Check sheet for the modelled part. Datum: model origin and axes. Units: mm. Face numbers are marked on the shaded views. A direction names the side the tool comes from. Round coordinates to 2 decimals unless told otherwise and drop trailing zeros. Write each loop counter-clockwise with the first axis right and the second up, starting at its lowest first coordinate (ties: lowest second). Pieces come first, ordered by that corner, then holes.
Item 1: Cross-section at B-B on y = -6.5. Enter the section's corners in (x, z).
Item 2: Tool access check on the marked faces 4, 5 and 6. Record the directions out of +Z, -Z, +X, -X, +Y, -Y that give a thin tool (end or side, any length) a straight path to the whole face; none if there is none.
Item 3: Release check for a two-part mould opening along X. For the marked faces 1, 2 and 3 record: +X half, -X half, draft (parallel to the pull), parting line (faces both ways), or undercut.
Item 4: Material ranges on line 1 (Z direction, x = -17.5, y = -27.55); line 2 (X direction, y = 25.5, z = 24); line 3 (X direction, y = -27, z = -8), recorded low to high.
Item 5: Go/stop test with flat-tipped pins: pin 1 Ø7.5 at (x, z) = (-17.5, 26.5) entering from +Y; pin 2 Ø8 at (x, y) = (20, 17) entering from -Z; pin 3 Ø4 at (x, z) = (13.5, 1) entering from +Y. Record where each tip stops, or that it passes through.
Item 6: Cross-section at C-C on z = 26.5. Enter the section's corners in (x, y), plus the area to 3 significant figures.
Item 7: Cross-section at D-D on x = 28.5. Enter the section's corners in (y, z).
Item 8: Cross-section at A-A on x = 17.5. Enter the section's corners in (y, z), plus the area to 3 significant figures.
from build123d import *

# Parameters (mm, degrees)
EXTRUDE_1_DEPTH     = 40
SKETCH_2_W          = 60
SKETCH_2_H          = 41.476322839
EXTRUDE_2_DEPTH     = 2.5
SKETCH_3_R          = 3.25
CUT_EXTRUDE_1_DEPTH = 10


with BuildPart() as part:
    # 草图1 → 凸台-拉伸1 (new, symmetric)
    with BuildSketch(Plane.XY):
        Polygon((-30, 30), (-30, -25), (30, -25), (30, 30), (35, 30), (35, -30), (-35, -30), (-35, 30), align=None)
    extrude(amount=EXTRUDE_1_DEPTH, both=True)

    # 草图2 → 凸台-拉伸2 (add, symmetric)
    with BuildSketch(Plane.XY):
        with Locations((0, -4.26183858)):
            Rectangle(SKETCH_2_W, SKETCH_2_H)
    extrude(amount=EXTRUDE_2_DEPTH, both=True)

    # 草图3 → 切除-拉伸1 (cut)
    with BuildSketch(Plane.XZ.offset(30)):
        with Locations((17.5, 26.5)):
            Circle(SKETCH_3_R)
        with Locations((17.5, -8.5)):
            Circle(SKETCH_3_R)
        with Locations((-17.5, -8.5)):
            Circle(SKETCH_3_R)
        with Locations((-17.5, 26.5)):
            Circle(SKETCH_3_R)
    extrude(amount=-CUT_EXTRUDE_1_DEPTH, mode=Mode.SUBTRACT)


solid = part.part
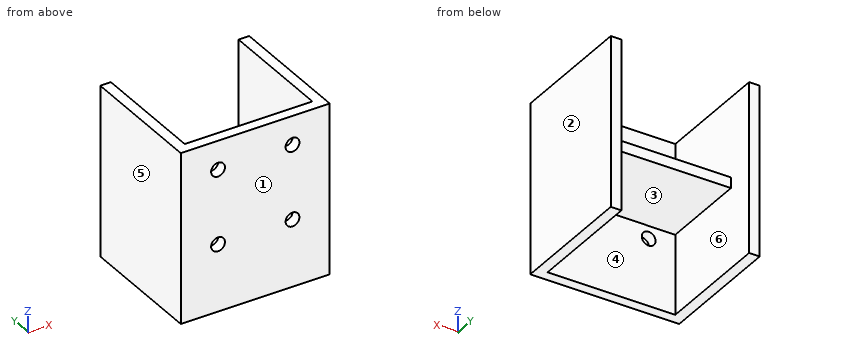
Response values:
1. outline: (-35, -40) - (-30, -40) - (-30, -2.5) - (30, -2.5) - (30, -40) - (35, -40) - (35, 40) - (30, 40) - (30, 2.5) - (-30, 2.5) - (-30, 40) - (-35, 40) - close
2. face 4: -Z, +Y
2. face 5: +Z, -Z, -X, +Y, -Y
2. face 6: +Y
3. face 1: draft
3. face 2: +X half
3. face 3: undercut
4. line 1: z = -40 to -11.75, -5.25 to 23.25, 29.75 to 40
4. line 2: x = -35 to -30, 30 to 35
4. line 3: x = -35 to -20.71, -14.29 to 14.29, 20.71 to 35
5. pin 1: stops at y = -25
5. pin 2: stops at z = -2.5
5. pin 3: stops at y = 16.48
6. outline: (-35, -30) - (-20.75, -30) - (-20.75, -25) - (-30, -25) - (-30, 30) - (-35, 30) - close; (-14.25, -30) - (14.25, -30) - (14.25, -25) - (-14.25, -25) - close; (20.75, -30) - (35, -30) - (35, 30) - (30, 30) - (30, -25) - (20.75, -25) - close
6. area: 835 mm2
7. outline: (-30, -40) - (-25, -40) - (-25, -2.5) - (16.48, -2.5) - (16.48, 2.5) - (-25, 2.5) - (-25, 40) - (-30, 40) - close
8. outline: (-30, -40) - (-25, -40) - (-25, -11.75) - (-30, -11.75) - close; (-30, -5.25) - (-25, -5.25) - (-25, -2.5) - (16.48, -2.5) - (16.48, 2.5) - (-25, 2.5) - (-25, 23.25) - (-30, 23.25) - close; (-30, 29.75) - (-25, 29.75) - (-25, 40) - (-30, 40) - close
8. area: 542 mm2
